Input: part model. Units: mm. Frame: model coordinates. Face numbers are marked on the shaded views. Coordinates: 2 decimals unless noted, no trailing zeros. Write each loop counter-clockwise with the first axis right and the second up, starting at its lowest first coordinate (ties: lowest second). Pieces come first, ordered by that corner, then holes. Notation, with made-up numbers: (76.25, 66.25) - (124.25, 66.25) arc R31 cw to (124.25, 93.25) - close; hole circle Ø6 at (-19, 83). An arc over 180 degrees is marked (long way). Use a Markdown table: item, result. Add a question column.
Q1. Section query C-C (z = 8.5). Return the cut outline in (x, y), then the cut area to 3 significant figures.
Q2. Section query D-D (x = 92). Return the cut outline in (y, z), then the cut area to 3 significant figures.
Q3. Material intervals for probe 1 along Y at (x, z) = (115, 6.75); probe 2 along Z at (x, y) = (113.5, -4.5); probe 3 along Y at (x, z) = (93, 6), sorted ascending. Write a range as from..to.
Q4. Mould query, pull axis X, two halves, no side actions, for the marked faces 1, 2, 3 and 4. Classes: released by +X, released by -X, zero draft, split by the parting line, or undercut.
Q5. Section query A-A (y = 0). Return the cut outline in (x, z), then the cut area to 3 significant figures.
Q6. Section query B-B (x = 117). Return the cut outline in (y, z).
Q7. Pin query (flat end, axial travel): P1, Ø4, axis at x = 115, y = 0, coming from the -Z side; P2, Ø1, axis at x = 95.5, z = 14.5, coming from the -Y side; P3, Ø6, axis at x = 108.5, y = -9, coming from the -Z side; P4, Ø8, axis at y = 34, z = 4, coming from the -X side. Return the tip coordinate at first contact, or that it passes through.
from build123d import *

# Parameters (mm, degrees)
EXTRUDE_1_DEPTH = 18
SKETCH_8_R      = 3.5
EXTRUDE_5_DEPTH = 5


with BuildPart() as part:
    # 草图1 → 凸台-拉伸1 (new body)
    with BuildSketch(Plane.XY):
        with BuildLine():
            Line((86.602540378, 50), (90.932667397, 52.5))
            ThreePointArc((90.932667397, 52.5), (105, 0), (90.932667397, -52.5))
            Line((90.932667397, -52.5), (86.602540378, -50))
            ThreePointArc((86.602540378, -50), (100, 0), (86.602540378, 50))
        make_face()
    extrude(amount=EXTRUDE_1_DEPTH)

    # 草图8 → 凸台-拉伸5 (add, symmetric)
    with BuildSketch(Plane.XY.offset(9)):
        with BuildLine():
            Line((103.468607759, 5.878851187), (102.726389869, -8.907444453))
            ThreePointArc((102.726389869, -8.907444453), (108.287042552, -7.083213633), (114.137686614, -6.946683786))
            ThreePointArc((114.137686614, -6.946683786), (121.944727548, 0.877928973), (112.436089109, 6.513552099))
            ThreePointArc((112.436089109, 6.513552099), (108.00101592, 5.508594665), (103.468607759, 5.878851187))
        make_face()
        with Locations((115, 0)):
            Circle(SKETCH_8_R, mode=Mode.SUBTRACT)
    extrude(amount=EXTRUDE_5_DEPTH, both=True)


solid = part.part
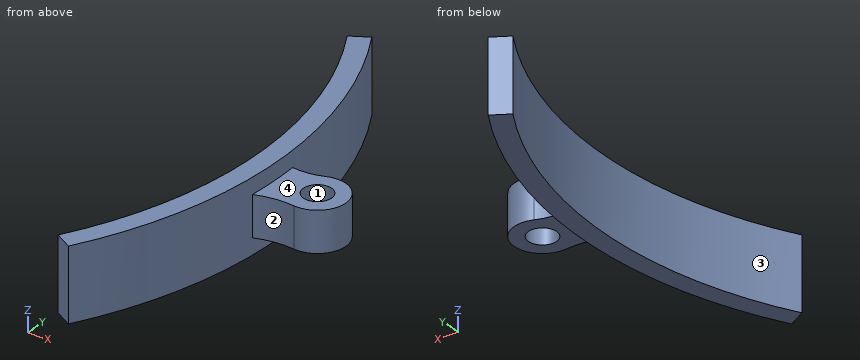
Values follow:
| question | item | result |
|---|---|---|
| 1 | outline | (86.6, -50) - (90.93, -52.5) arc R105 ccw to (104.69, -8.05) arc R20 cw to (114.14, -6.95) arc R7 ccw (long way) to (112.44, 6.51) arc R15 cw to (104.85, 5.62) arc R105 ccw to (90.93, 52.5) - (86.6, 50) arc R100 cw to start; hole circle Ø7 at (115, 0) |
| 1 | area | 707 mm2 |
| 2 | outline | (-50.61, 0) - (-39.19, 0) - (-39.19, 18) - (-50.61, 18) - close; (39.19, 0) - (50.61, 0) - (50.61, 18) - (39.19, 18) - close |
| 2 | area | 411 mm2 |
| 3 | probe 1 | -7..-3.5, 3.5..7 |
| 3 | probe 2 | 4..14 |
| 3 | probe 3 | -48.74..-36.76, 36.76..48.74 |
| 4 | face 1 | undercut |
| 4 | face 2 | undercut |
| 4 | face 3 | released by -X |
| 4 | face 4 | zero draft |
| 5 | outline | (100, 0) - (105, 0) - (105, 4) - (111.5, 4) - (111.5, 14) - (105, 14) - (105, 18) - (100, 18) - close; (118.5, 4) - (122, 4) - (122, 14) - (118.5, 14) - close |
| 5 | area | 190 mm2 |
| 6 | outline | (-6.71, 4) - (-2.87, 4) - (-2.87, 14) - (-6.71, 14) - close; (2.87, 4) - (6.71, 4) - (6.71, 14) - (2.87, 14) - close |
| 7 | P1 | through |
| 7 | P2 | y = -44.72 |
| 7 | P3 | z = 4 |
| 7 | P4 | x = 92.5 |
